Job drawing, mm, ordinate dimensions from the low corner. One solid piece. Round coordinates to 2 decimals unless told otherwise and drop trailing zeros. Loops run counter-clockwise (first coordinate to the right, second up) from the corner with the lowest first, then second, coordinate; pieces in that order, holes last. Notation, with made-up numbers: M 73.25,-25 L 92.25,-25 A9 ccw 92.25,-14 Z; hole C -23.75,50 d9. An arc over 180 degrees is marked long. One line per item, written item: value.
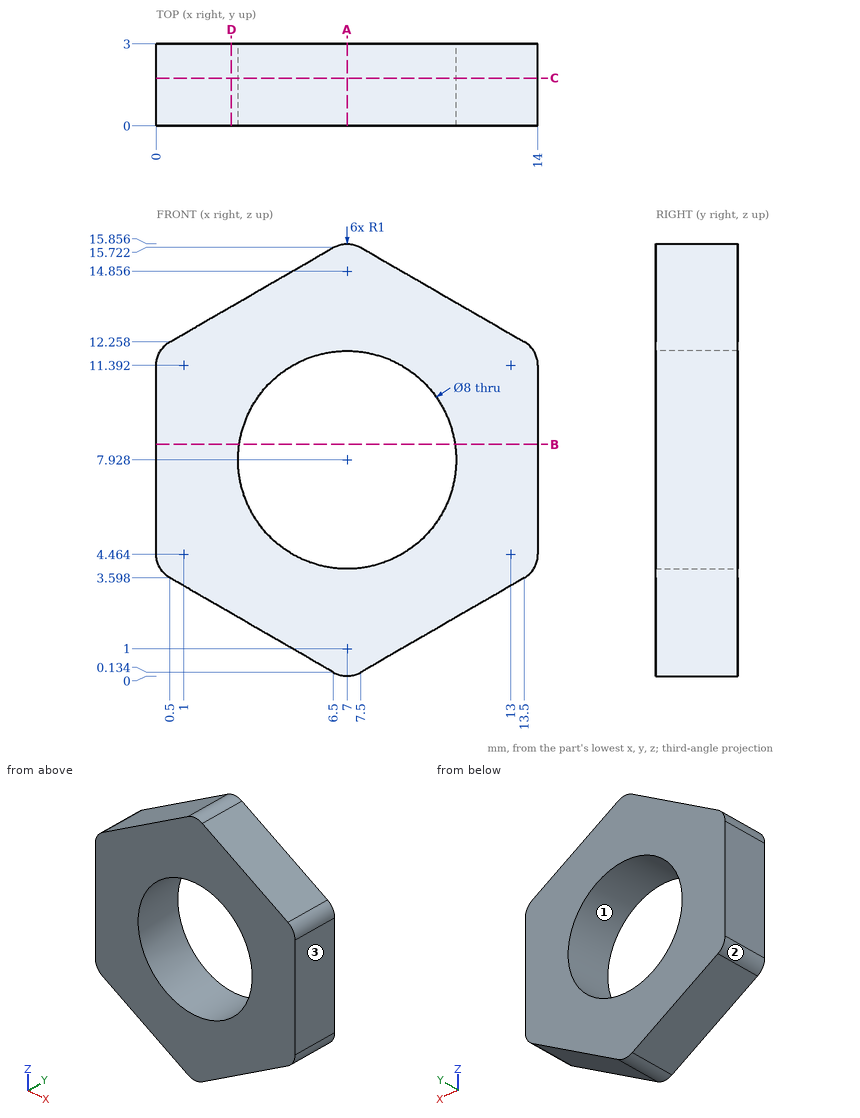
Item 1: Slice it at A-A, the plane x = 7. Give the cut face in (y, z).
Check values:
outline: M 0,0 L 3,0 L 3,3.93 L 0,3.93 Z; M 0,11.93 L 3,11.93 L 3,15.86 L 0,15.86 Z
Item 2: Drop a flat-ended pin along its axis: P1, Ø1.5, axis at x = 4.5, y = 2.5, coming from the +Z side. Give the stop position or say it passes through.
Check values:
P1: stops at z = 15
Item 3: Pull direction X, two halves, no side cores. Call the marked faces 1, 2 and 3: pulls with the +X half, pulls with the -X half, needs draft (parallel to the pull), parting line crosses it, or undercut.
Check values:
face 1: undercut
face 2: pulls with the -X half
face 3: pulls with the +X half
Item 4: Slice it at C-C, the plane y = 1.75. Give the cut face in (x, z), and give its area (3 significant figures).
Check values:
outline: M 0,4.46 A1 ccw 0.5,3.6 L 6.5,0.13 A1 ccw 7.5,0.13 L 13.5,3.6 A1 ccw 14,4.46 L 14,11.39 A1 ccw 13.5,12.26 L 7.5,15.72 A1 ccw 6.5,15.72 L 0.5,12.26 A1 ccw 0,11.39 Z; hole C 7,7.93 d8
area: 119 mm2
Item 5: Slice it at D-D, the plane x = 2.75. Give the cut face in (y, z).
Check values:
outline: M 0,2.3 L 3,2.3 L 3,13.56 L 0,13.56 Z
Item 6: Slice it at B-B, the plane z = 8.5. Give the cut face in (x, y).
Check values:
outline: M 0,0 L 3.04,0 L 3.04,3 L 0,3 Z; M 10.96,0 L 14,0 L 14,3 L 10.96,3 Z
Item 7: Wall check: line 1 along X through (y, z) = (0.75, 11) (1 decimal); line 2 along X through (y, z) = (2.1, 7.75); line 3 along X through (y, z) = (0.5, 12) (1 decimal). Give the ranges that are in metal, low to high.
Check values:
line 1: x = 0 to 4.4, 9.6 to 14
line 2: x = 0 to 3, 11 to 14
line 3: x = 0.2 to 13.8
